from build123d import *

# Parameters (mm, degrees)
SKETCH1_R          = 5
SKETCH1_R_2        = 4
BOSS_EXTRU_1_DEPTH = 7.9
SKETCH2_R          = 5
CUT_EXTRUDE1_DEPTH = 212.826281623
FILLET1_R          = 10


with BuildPart() as part:
    # Sketch1 → Boss.-Extru.1 (new body)
    with BuildSketch(Plane(origin=(0, 0, 0), x_dir=(1, 0, 0), z_dir=(0, 1, 0))):
        with BuildLine():
            Line((149.698750242, -34.853527415), (116.932668471, -11.910469961))
            ThreePointArc((116.932668471, -11.910469961), (108.746549365, -7.873522768), (99.72537538, -6.48503129))
            Line((99.72537538, -6.48503129), (9.72537538, -6.48503129))
            ThreePointArc((9.72537538, -6.48503129), (2.654307568, -9.413963478), (-0.27462462, -16.48503129))
            Line((-0.27462462, -16.48503129), (-0.27462462, -76.48503129))
            Line((-0.27462462, -76.48503129), (-30.27462462, -76.48503129))
            Line((-30.27462462, -76.48503129), (-30.27462462, -4.017204085))
            ThreePointArc((-30.27462462, -4.017204085), (-21.487828056, 17.195999351), (-0.27462462, 25.982795915))
            Line((-0.27462462, 25.982795915), (105.659916542, 25.982795915))
            ThreePointArc((105.659916542, 25.982795915), (114.681090527, 24.594304438), (122.867209633, 20.557357244))
            Line((122.867209633, 20.557357244), (196.395516927, -30.927717795))
            Line((196.395516927, -30.927717795), (197.377819359, -36.498631718))
            Line((197.377819359, -36.498631718), (190.606283823, -46.169386696))
            Line((190.606283823, -46.169386696), (184.570257854, -48.031947572))
            Line((184.570257854, -48.031947572), (149.698750242, -34.853527415))
        make_face()
        with Locations(Location((188.311978078, -34.853527415, 0), (0, 0, 270))):
            Circle(SKETCH1_R, mode=Mode.SUBTRACT)
        with Locations(Location((-15.27462462, -69.11920583, 0), (0, 0, 270))):
            Circle(SKETCH1_R_2, mode=Mode.SUBTRACT)
    extrude(amount=BOSS_EXTRU_1_DEPTH)

    # Sketch2 → Cut-Extrude1 (cut, through all)
    with BuildSketch(Plane.XZ):
        with Locations(Location((114.715355874, -1.93178017, 0), (0, 0, 270))):
            Circle(SKETCH2_R)
    extrude(amount=-CUT_EXTRUDE1_DEPTH, mode=Mode.SUBTRACT)

    # Fillet1
    fillet1_edges = [part.edges().sort_by_distance(p)[0] for p in [
        (-30.27462462, 3.95, 76.48503129),
        (-0.27462462, 3.95, 76.48503129),
    ]]
    fillet(fillet1_edges, radius=FILLET1_R)


solid = part.part
Geometry check sheet. Reference: the model listing, model coordinates, mm. A direction names the side the tool comes from. Give positions to 0.01 mm unless a question says otherwise; leave off trailing zeros. Order: outer loops, then holes, each group sorted by start corner. A loop starts at its lowest first (then second) coordinate and runs counter-clockwise, first axis right, second up.
1) Cross-section at C-C (x = 31). Record the boundary of the cut face in (y, z), then the cut area to 3 significant figures.
Results are:
outline: (0, -25.98) - (7.9, -25.98) - (7.9, 6.49) - (0, 6.49) - close
area: 256 mm2
2) Tool access check on faces 1 (the cylindrical face through (193.27, 3.89, 34.2)), 2 (the flat face through (55, 4, 6.485)). Record the directions out of +Z, -Z, +X, -X, +Y, -Y that give a thin tool (end or side, any length) a straight path to the whole face; none if there is none.
Results are:
face 1: +Y, -Y
face 2: +Z, +Y, -Y
3) Cross-section at A-A (z = 20). Record the boundary of the cut face in (x, y).
Results are:
outline: (-30.27, 0) - (-0.27, 0) - (-0.27, 7.9) - (-30.27, 7.9) - close; (128.49, 0) - (180.79, 0) - (180.79, 7.9) - (128.49, 7.9) - close
4) Cross-section at B-B (y = 5.5). Record the boundary of the cut face in (x, z).
Results are:
outline: (-30.27, 4.02) arc R30 ccw to (-0.27, -25.98) - (105.66, -25.98) arc R30 ccw to (122.87, -20.56) - (196.4, 30.93) - (197.38, 36.5) - (190.61, 46.17) - (184.57, 48.03) - (149.7, 34.85) - (116.93, 11.91) arc R30 cw to (99.73, 6.49) - (9.73, 6.49) arc R10 cw to (-0.27, 16.49) - (-0.27, 66.49) arc R10 ccw to (-10.27, 76.49) - (-20.27, 76.49) arc R10 ccw to (-30.27, 66.49) - close; hole circle Ø8 at (-15.27, 69.12); hole circle Ø10 at (114.72, -1.93); hole circle Ø10 at (188.31, 34.85)
5) Draft check along Z on faces 3 (the cylindrical face through (-11.31, 3.89, 68.6)), 4 (the flat face through (196.88, 3.89, 33.67)), 5 (the cylindrical face through (108.869, 3.895, 7.912)). Enter one of: released by +Z, released by -Z, zero draft, split by the parting line, or undercut.
Results are:
face 3: undercut
face 4: released by -Z
face 5: released by +Z
6) Cross-section at D-D (z = -0.5). Record the boundary of the cut face in (x, y), then the cut area to 3 significant figures.
Results are:
outline: (-29.93, 0) - (109.92, 0) - (109.92, 7.9) - (-29.93, 7.9) - close; (119.51, 0) - (151.51, 0) - (151.51, 7.9) - (119.51, 7.9) - close
area: 1,360 mm2
7) Material ranges on probe 1 along X at (y, z) = (3.75, 51.5); probe 2 along Z at (x, y) = (93, 2); probe 3 along X at (y, z) = (3.75, 9), recorded low to high.
Results are:
probe 1: x = -30.27 to -0.27
probe 2: z = -25.98 to 6.49
probe 3: x = -30.27 to 3.09, 111.75 to 165.08
8) Gauge pin test, flat ends, axial feed: pin 1 (8 mm diameter, centred on x = 188.31, z = 34.85, fed in from +Y); pin 2 (4 mm diameter, centred on x = 132, y = 4, fed in from -Z); pin 3 (1.5 mm diameter, centred on y = 6.5, z = 53.5, fed in from +X); pin 4 (2.5 mm diameter, centred on x = 73, y = 6, fed in from +Z). Record the tip position at first contact, or that the pin passes through.
Results are:
pin 1: passes through
pin 2: stops at z = -15.56
pin 3: stops at x = -0.27
pin 4: stops at z = 6.49
